Geometry check sheet. Reference: drawing and pictorial views, mm from the part's lowest x, y, z. Round coordinates to 2 decimals unless told otherwise and drop trailing zeros. Order: outer loops, then holes, each group sorted by start corner. A loop starts at its lowest first (then second) coordinate and runs counter-clockwise, first axis right, second up.
(1) Material ranges on line 1 along Y through (x, z) = (40, 3.25); line 2 along X through (y, z) = (60, 7.5); line 3 along Y through (x, z) = (42, 9.5), recorded low to high.
(2) Release check for a two-part mould opening along X. For the marked faces 1, 2 and 3 record: +X half, -X half, draft (parallel to the pull), parting line (faces both ways), or undercut.
(3) Sectioned sample at B-B (z = 4.75). Record the boundary of the cut face in (x, y), plus the area to 3 significant figures.
(4) Sectioned sample at A-A (y = 20). Record the boundary of the cut face in (x, z) (3 decimals).
(5) Sectioned sample at C-C (x = 40). Record the boundary of the cut face in (y, z) (3 decimals), plus the area to 3 significant figures.
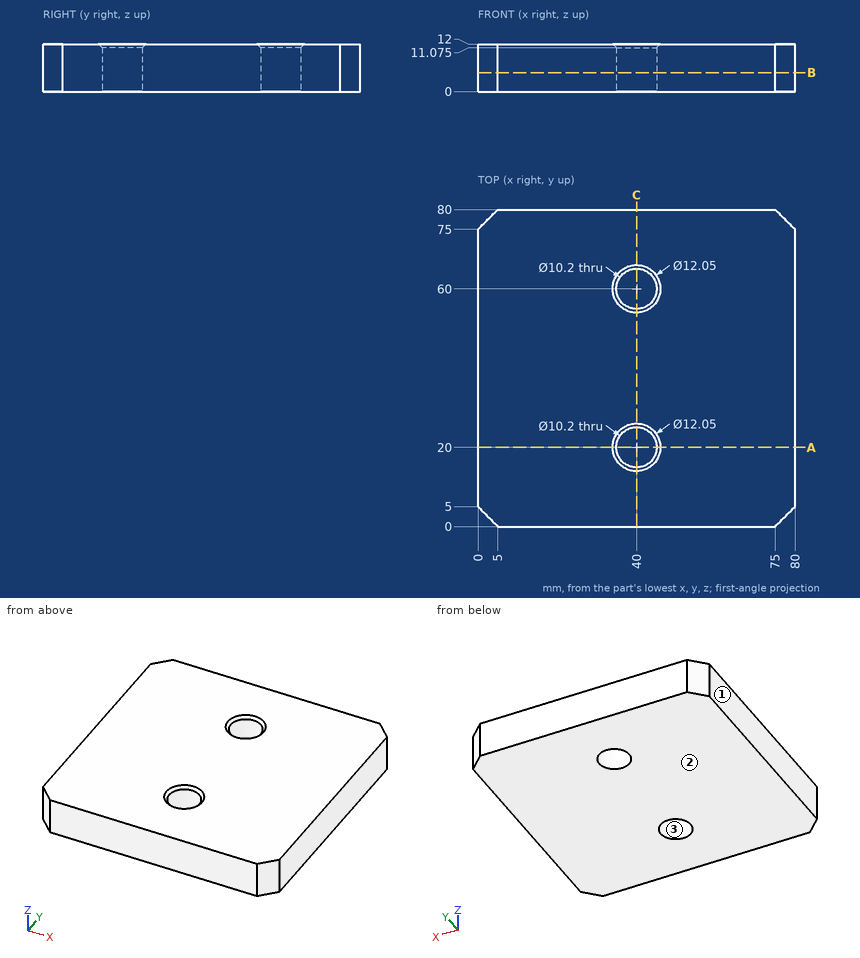
Answer below:
1. line 1: y = 0 to 14.9, 25.1 to 54.9, 65.1 to 80
1. line 2: x = 0 to 34.9, 45.1 to 80
1. line 3: y = 0 to 15.31, 24.69 to 55.31, 64.69 to 80
2. face 1: -X half
2. face 2: draft
2. face 3: undercut
3. outline: (0, 5) - (5, 0) - (75, 0) - (80, 5) - (80, 75) - (75, 80) - (5, 80) - (0, 75) - close; hole circle Ø10.2 at (40, 20); hole circle Ø10.2 at (40, 60)
3. area: 6,190 mm2
4. outline: (0, 0) - (34.9, 0) - (34.9, 11.075) - (33.975, 12) - (0, 12) - close; (45.1, 0) - (80, 0) - (80, 12) - (46.025, 12) - (45.1, 11.075) - close
5. outline: (0, 0) - (14.9, 0) - (14.9, 11.075) - (13.975, 12) - (0, 12) - close; (25.1, 0) - (54.9, 0) - (54.9, 11.075) - (53.975, 12) - (26.025, 12) - (25.1, 11.075) - close; (65.1, 0) - (80, 0) - (80, 12) - (66.025, 12) - (65.1, 11.075) - close
5. area: 713 mm2
